Geometry check sheet. Reference: the model listing, model coordinates, mm. Round coordinates to 2 decimals unless told otherwise and drop trailing zeros. Loops run counter-clockwise (first coordinate to the right, second up) from the corner with the lowest first, then second, coordinate; pieces in that order, holes last. Notation, with made-up numbers: (49, 14.25) -> (81, 14.25) arc R27 cw to (81, 40.25) -> close; hole circle Ø6 at (37.25, 31). An arc over 180 degrees is marked (long way). Use a Markdown table: item, result. Add a question column.
Q1. Sectioned sample at A-A, the plane x = 60. Enter the section's corners in (y, z), then the cut area to 3 significant figures.
Q2. Gauge pin test, flat end, axial feed: P1, Ø6.5, axis at x = 60, y = 10, coming from the +Z side. Record the tip position at first contact, or that the pin passes through.
Q3. Release check for a two-part mould opening along Y. For faces 1 (the face through (-63.497, 10.154, 2.535)), 2 (the face through (70, -3, 2)), 3 (the face through (56.503, 10.154, 2.535)), 4 (the face through (-1, -20, 2)) record: released by +Y, released by -Y, zero draft, split by the parting line, or undercut.
Q4. Sectioned sample at C-C, the plane z = 3. Enter the section's corners in (x, y).
Q5. Material ranges on L1, parallel to Y at x = -60, z = 2.3; L2, parallel to X at y = 10.5, z = 1.85; L3, parallel to X at y = 13, z = 2.15, recorded low to high.
Q6. Sectioned sample at B-B, the plane y = 10. Enter the section's corners in (x, z).
```python
from build123d import *

# Parameters (mm, degrees)
SKETCH_1_W          = 140
SKETCH_1_H          = 40
EXTRUDE_1_DEPTH     = 5
SKETCH_2_R          = 3.5
CUT_EXTRUDE_1_DEPTH = 5
CHAMFER_1_SIZE      = 5


with BuildPart() as part:
    # 草图1 → 凸台-拉伸1 (new body)
    with BuildSketch(Plane.XY):
        Rectangle(SKETCH_1_W, SKETCH_1_H)
    extrude(amount=EXTRUDE_1_DEPTH)

    # 草图2 → 切除-拉伸1 (cut)
    with BuildSketch(Plane.XY.offset(5)):
        with Locations((-60, 10)):
            Circle(SKETCH_2_R)
        with Locations((60, 10)):
            Circle(SKETCH_2_R)
    extrude(amount=-CUT_EXTRUDE_1_DEPTH, mode=Mode.SUBTRACT)

    # 倒角1
    chamfer_1_edges = [part.edges().sort_by_distance(p)[0] for p in [
        (-70, 20, 2.5),
        (70, 20, 2.5),
    ]]
    chamfer(chamfer_1_edges, length=CHAMFER_1_SIZE)


solid = part.part
```
Values:
| question | item | result |
|---|---|---|
| 1 | outline | (-20, 0) -> (6.5, 0) -> (6.5, 5) -> (-20, 5) -> close; (13.5, 0) -> (20, 0) -> (20, 5) -> (13.5, 5) -> close |
| 1 | area | 165 mm^2 |
| 2 | P1 | through |
| 3 | face 1 | undercut |
| 3 | face 2 | zero draft |
| 3 | face 3 | undercut |
| 3 | face 4 | released by -Y |
| 4 | outline | (-70, -20) -> (70, -20) -> (70, 15) -> (65, 20) -> (-65, 20) -> (-70, 15) -> close; hole circle Ø7 at (-60, 10); hole circle Ø7 at (60, 10) |
| 5 | L1 | -20 to 6.5, 13.5 to 20 |
| 5 | L2 | -70 to -63.46, -56.54 to 56.54, 63.46 to 70 |
| 5 | L3 | -70 to -61.8, -58.2 to 58.2, 61.8 to 70 |
| 6 | outline | (-70, 0) -> (-63.5, 0) -> (-63.5, 5) -> (-70, 5) -> close; (-56.5, 0) -> (56.5, 0) -> (56.5, 5) -> (-56.5, 5) -> close; (63.5, 0) -> (70, 0) -> (70, 5) -> (63.5, 5) -> close |
